Geometry: final body of the model. Coordinates: model frame, mm. Face numbers are marked on the shaded views. A direction names the side the tool comes from. Give positions to 0.01 mm unless a question says otherwise; leave off trailing zeros. Loops run counter-clockwise (first coordinate to the right, second up) from the corner with the lowest first, then second, coordinate; pieces in that order, holes last.
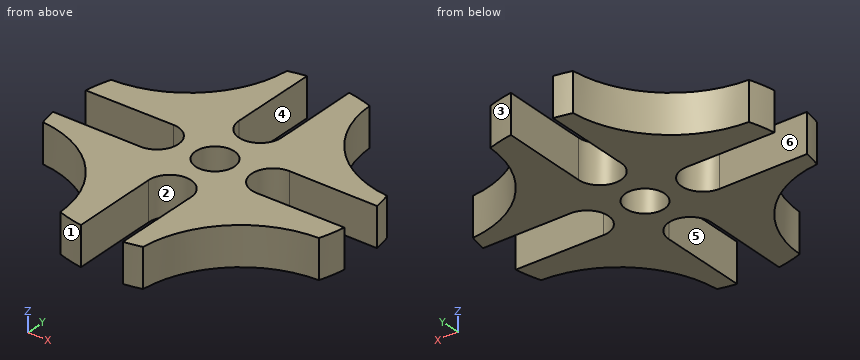
from build123d import *

# Parameters (mm, degrees)
GENEVA_WHEEL_PROFILE_R       = 5
GENEVA_WHEEL_BODY_10MM_DEPTH = 10


with BuildPart() as part:
    # Geneva Wheel Profile → Geneva Wheel Body 10mm (new body)
    with BuildSketch(Plane.XY):
        with BuildLine():
            ThreePointArc((-36.078505425, 11.862749321), (-18.305680685, 19.283646977), (-10, 36.66060556))
            ThreePointArc((-10, 36.66060556), (-7.764216189, 37.198346025), (-5.5, 37.599867021))
            Line((-5.5, 37.599867021), (-5.5, 15))
            ThreePointArc((-5.5, 15), (0, 9.5), (5.5, 15))
            Line((5.5, 15), (5.350081788, 37.6))
            ThreePointArc((5.350081788, 37.6), (8.639972519, 36.982891315), (11.862749321, 36.078505425))
            ThreePointArc((11.862749321, 36.078505425), (19.283646977, 18.305680685), (36.66060556, 10))
            ThreePointArc((36.66060556, 10), (37.198346025, 7.764216189), (37.599867021, 5.5))
            Line((37.599867021, 5.5), (15, 5.5))
            ThreePointArc((15, 5.5), (9.5, 0), (15, -5.5))
            Line((15, -5.5), (37.6, -5.350081788))
            ThreePointArc((37.6, -5.350081788), (36.982891315, -8.639972519), (36.078505425, -11.862749321))
            ThreePointArc((36.078505425, -11.862749321), (18.305680685, -19.283646977), (10, -36.66060556))
            ThreePointArc((10, -36.66060556), (7.764216189, -37.198346025), (5.5, -37.599867021))
            Line((5.5, -37.599867021), (5.5, -15))
            ThreePointArc((5.5, -15), (0, -9.5), (-5.5, -15))
            Line((-5.5, -15), (-5.350081788, -37.6))
            ThreePointArc((-5.350081788, -37.6), (-8.639972519, -36.982891315), (-11.862749321, -36.078505425))
            ThreePointArc((-11.862749321, -36.078505425), (-19.283646977, -18.305680685), (-36.66060556, -10))
            ThreePointArc((-36.66060556, -10), (-37.198346025, -7.764216189), (-37.599867021, -5.5))
            Line((-37.599867021, -5.5), (-15, -5.5))
            ThreePointArc((-15, -5.5), (-9.5, 0), (-15, 5.5))
            Line((-15, 5.5), (-37.6, 5.350081788))
            ThreePointArc((-37.6, 5.350081788), (-36.982891315, 8.639972519), (-36.078505425, 11.862749321))
        make_face()
        Circle(GENEVA_WHEEL_PROFILE_R, mode=Mode.SUBTRACT)
    extrude(amount=GENEVA_WHEEL_BODY_10MM_DEPTH)


solid = part.part
Item 1: Pin query (flat end, axial travel): pin 1 (2 mm diameter, centred on y = -14, z = 8.5, fed in from -X); pin 2 (1 mm diameter, centred on y = -22.5, z = 2.5, fed in from +X); pin 3 (4 mm diameter, centred on x = -24, z = 8.5, fed in from -Y). Return the tip coordinate at first contact, or that it passes through.
Values follow:
pin 1: stops at x = -26.31
pin 2: stops at x = 15.81
pin 3: stops at y = -15.81
Item 2: Set-up query: the marked faces 4, 5 and 6. Return all of +Z, -Z, +X, -X, +Y, -Y with unobstructed straight access to the full face (end or side cutting, diameter ignored); none if empty.
Values follow:
face 4: +Z, -Z, +Y
face 5: +Z, -Z, -Y
face 6: +Z, -Z, -X
Item 3: Ray query, probe 1 along Y at (x, z) = (0, 2.75); probe 2 along X at (y, z) = (-26.5, 2.5); probe 3 along Y at (x, z) = (3.5, 1.5). Return the intervals inside material, ascending.
Values follow:
probe 1: y = -9.5 to -5, 5 to 9.5
probe 2: x = -13.94 to -5.42, 5.5 to 12.9
probe 3: y = -10.76 to -3.57, 3.57 to 10.76
Item 4: Section query C-C on z = 3.5. Return loops of the section in (x, y).
Values follow:
outline: (-37.6, -5.5) arc R38 ccw to (-36.66, -10) arc R27 cw to (-11.86, -36.08) arc R37.98 ccw to (-5.35, -37.6) - (-5.5, -15) arc R5.5 cw to (5.5, -15) - (5.5, -37.6) arc R38 ccw to (10, -36.66) arc R27 cw to (36.08, -11.86) arc R37.98 ccw to (37.6, -5.35) - (15, -5.5) arc R5.5 cw to (15, 5.5) - (37.6, 5.5) arc R38 ccw to (36.66, 10) arc R27 cw to (11.86, 36.08) arc R37.98 ccw to (5.35, 37.6) - (5.5, 15) arc R5.5 cw to (-5.5, 15) - (-5.5, 37.6) arc R38 ccw to (-10, 36.66) arc R27 cw to (-36.08, 11.86) arc R37.98 ccw to (-37.6, 5.35) - (-15, 5.5) arc R5.5 cw to (-15, -5.5) - close; hole circle Ø10 at (0, 0)
Item 5: Section query A-A on x = 0. Return loops of the section in (y, z).
Values follow:
outline: (-9.5, 0) - (-5, 0) - (-5, 10) - (-9.5, 10) - close; (5, 0) - (9.5, 0) - (9.5, 10) - (5, 10) - close
Item 6: Draft query along X for the marked faces 1, 2 and 3. Return one class per face: +X half, -X half, draft (parallel to the pull), parting line (faces both ways), or undercut.
Values follow:
face 1: -X half
face 2: undercut
face 3: +X half
